from build123d import *

# Parameters (mm, degrees)
SKETCH1_W           = 152.4
SKETCH1_H           = 377.95
SKETCH1_R           = 11.125
BOSS_EXTRUDE1_DEPTH = 14


with BuildPart() as part:
    # Sketch1 → Boss-Extrude1 (new body)
    with BuildSketch(Plane.XY):
        Rectangle(SKETCH1_W, SKETCH1_H)
        with Locations((-57.15, 169.8625)):
            Circle(SKETCH1_R, mode=Mode.SUBTRACT)
        with Locations((57.15, 169.8625)):
            Circle(SKETCH1_R, mode=Mode.SUBTRACT)
        with Locations((57.15, -169.8625)):
            Circle(SKETCH1_R, mode=Mode.SUBTRACT)
        with Locations((-57.15, -169.8625)):
            Circle(SKETCH1_R, mode=Mode.SUBTRACT)
    extrude(amount=BOSS_EXTRUDE1_DEPTH)


solid = part.part
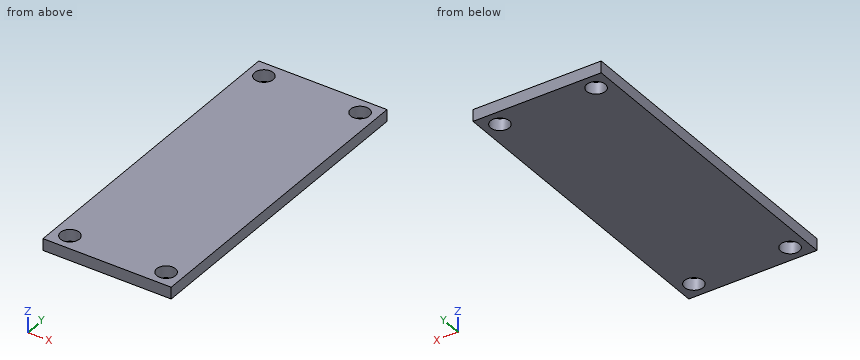
Work out the finished part from the listing and answer in its coordinate system (mm). Coordinates: 2 decimals unless noted, no trailing zeros. Write each loop counter-clockwise with the first axis right and the second up, starting at its lowest first coordinate (ties: lowest second). Pieces come first, ordered by that corner, then holes.
1. Flat-ended cylindrical pins translate along their axes: pin 1 (13.5 mm diameter, centred on x = -57.15, y = -169.86, fed in from +Z); pin 2 (10 mm diameter, centred on x = -43, y = 110.5, fed in from -Z). Find the tip coordinate at first contact, or state that the pin passes through.
Results list:
pin 1: passes through
pin 2: stops at z = 0
2. The part is cut by section B-B, the plane z = 3.75. State how many separate pieces and enclosed holes the cut face has, and give its area (3 significant figures).
Results list:
separate pieces: 1
enclosed holes: 4
area: 56,000 mm2
3. Consider line 1 along Y through (x, z) = (-57.15, 9) (1 decimal); line 2 along X through (y, z) = (-169.5, 9.5); line 3 along Y through (x, z) = (52, 3.25) (3 decimals). Determine where each line is inside the solid, lowest interval first.
Results list:
line 1: y = -189 to -181, -158.7 to 158.7, 181 to 189
line 2: x = -76.2 to -68.27, -46.03 to 46.03, 68.27 to 76.2
line 3: y = -188.975 to -179.724, -160.001 to 160.001, 179.724 to 188.975
4. The part is cut by section A-A, the plane x = 57.15. Write down the section's boundary in (y, z) (1 decimal), and give its area (3 significant figures).
Results list:
outline: (-189, 0) - (-181, 0) - (-181, 14) - (-189, 14) - close; (-158.7, 0) - (158.7, 0) - (158.7, 14) - (-158.7, 14) - close; (181, 0) - (189, 0) - (189, 14) - (181, 14) - close
area: 4,670 mm2
